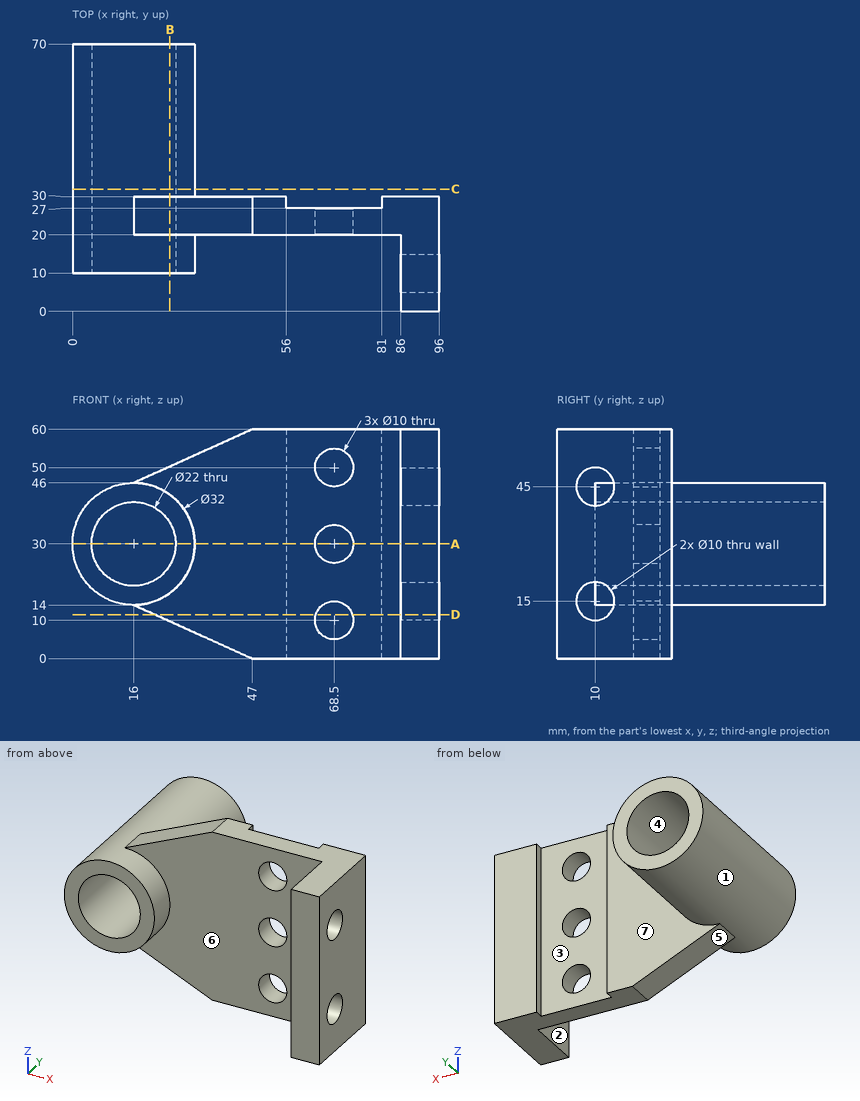
The drawing under review shows one solid part. Ordinate dimensions are in mm from its lowest x, y, z. A direction names the side the tool comes from. Coordinates: 2 decimals unless noted, no trailing zeros. Loops run counter-clockwise (first coordinate to the right, second up) from the corner with the lowest first, then second, coordinate; pieces in that order, holes last.
Item 1: Wall thickness on L1, parallel to X at y = 24, z = 30; L2, parallel to X at y = 36.5, z = 30; L3, parallel to Y at x = 73.5, z = 52.5: over which ranges is each line inside the solid? List them lowest first.
Completed:
L1: x = 0 to 5, 27 to 63.5, 73.5 to 96
L2: x = 0 to 5, 27 to 32
L3: y = 20 to 27
Item 2: Add section C-C (y = 32). Write out the cut boundary in (x, z), and give its area (3 significant figures).
Completed:
outline: circle Ø32 at (16, 30); hole circle Ø22 at (16, 30)
area: 424 mm2
Item 3: For the marked faces 1, 2 and 3, list the 3-axis set-ups (+Z, -Z, +X, -X, +Y, -Y) from which the entire face can be reached by the end or side of a thin tool; tool diameter is ignored.
Completed:
face 1: none
face 2: +Z, -Z, -Y
face 3: +Z, -Z, +Y
Item 4: Draft analysis for pull direction X (two halves, no side actions). For the marked faces 4, 5, 6 and 7, state which applies: pulls with the +X half, pulls with the -X half, needs draft (parallel to the pull), parting line crosses it, or undercut.
Completed:
face 4: undercut
face 5: pulls with the -X half
face 6: undercut
face 7: needs draft
Item 5: Add section B-B (x = 25.5). Write out the cut boundary in (y, z).
Completed:
outline: (10, 17.13) - (20, 17.13) - (20, 9.71) - (30, 9.71) - (30, 17.13) - (70, 17.13) - (70, 24.45) - (10, 24.45) - close; (10, 35.55) - (70, 35.55) - (70, 42.87) - (30, 42.87) - (30, 50.29) - (20, 50.29) - (20, 42.87) - (10, 42.87) - close
Item 6: Add section D-D (z = 11.5). Write out the cut boundary in (x, y), and give its area (3 significant figures).
Completed:
outline: (21.54, 20) - (63.73, 20) - (63.73, 27) - (56, 27) - (56, 30) - (21.54, 30) - close; (73.27, 20) - (86, 20) - (86, 13.57) - (96, 13.57) - (96, 30) - (81, 30) - (81, 27) - (73.27, 27) - close; (86, 0) - (96, 0) - (96, 6.43) - (86, 6.43) - close
area: 731 mm2
Item 7: Clearance check with flat-ended pins moving along their axes: pin 1 (13 mm diameter, centred on x = 68.5, z = 50, fed in from +Y); pin 2 (5 mm diameter, centred on x = 57.5, z = 21, fed in from +Y); pin 3 (2.5 mm diameter, centred on y = 29, z = 32, fed in from -X); pin 4 (8 mm diameter, centred on x = 68.5, z = 30, fed in from -Y). State where each tip first meets the part, or that it passes through.
Completed:
pin 1: stops at y = 27
pin 2: stops at y = 30
pin 3: stops at x = 0.02
pin 4: passes through
Item 8: Add section A-A (z = 30). Write out the cut boundary in (x, y), and give its area (4 significant figures).
Completed:
outline: (0, 10) - (5, 10) - (5, 70) - (0, 70) - close; (27, 10) - (32, 10) - (32, 20) - (63.5, 20) - (63.5, 27) - (56, 27) - (56, 30) - (32, 30) - (32, 70) - (27, 70) - close; (73.5, 20) - (86, 20) - (86, 0) - (96, 0) - (96, 30) - (81, 30) - (81, 27) - (73.5, 27) - close
area: 1,295 mm2
